from build123d import *

# Parameters (mm, degrees)
SKETCH_1_R          = 5.25
EXTRUDE_1_DEPTH     = 15
SKETCH_2_R          = 40
EXTRUDE_2_DEPTH     = 10
SKETCH_3_R          = 25
CUT_EXTRUDE_1_DEPTH = 113.805141727
FILLET_1_R          = 3


with BuildPart() as part:
    # 草图1 → 凸台-拉伸1 (new body)
    with BuildSketch(Plane.XY):
        with BuildLine():
            ThreePointArc((0, 77.781745931), (48.328171063, 48.328171063), (77.781745931, 0))
            ThreePointArc((77.781745931, 0), (48.328171063, -48.328171063), (0, -77.781745931))
            ThreePointArc((0, -77.781745931), (-48.328171063, -48.328171063), (-77.781745931, 0))
            ThreePointArc((-77.781745931, 0), (-48.328171063, 48.328171063), (0, 77.781745931))
        make_face()
        with Locations((0, 60)):
            Circle(SKETCH_1_R, mode=Mode.SUBTRACT)
        with Locations((60, 0)):
            Circle(SKETCH_1_R, mode=Mode.SUBTRACT)
        with Locations((0, -60)):
            Circle(SKETCH_1_R, mode=Mode.SUBTRACT)
        with Locations((-60, 0)):
            Circle(SKETCH_1_R, mode=Mode.SUBTRACT)
    extrude(amount=EXTRUDE_1_DEPTH)

    # 草图2 → 凸台-拉伸2 (add)
    with BuildSketch(Plane.XY.offset(15)):
        with Locations(Location((0, 0, 0), (0, 0, 180))):
            Circle(SKETCH_2_R)
    extrude(amount=EXTRUDE_2_DEPTH)

    # 草图3 → 切除-拉伸1 (cut, through all)
    with BuildSketch(Plane.XY.offset(25)):
        Circle(SKETCH_3_R)
    extrude(amount=-CUT_EXTRUDE_1_DEPTH, mode=Mode.SUBTRACT)

    # 圆角1
    fillet_1_edges = [part.edges().sort_by_distance(p)[0] for p in [
        (48.328171063, -48.328171063, 15),
        (48.328171063, 48.328171063, 15),
        (40, 0, 15),
        (40, 0, 25),
        (-48.328171063, 48.328171063, 15),
        (-48.328171063, -48.328171063, 15),
    ]]
    fillet(fillet_1_edges, radius=FILLET_1_R)


solid = part.part
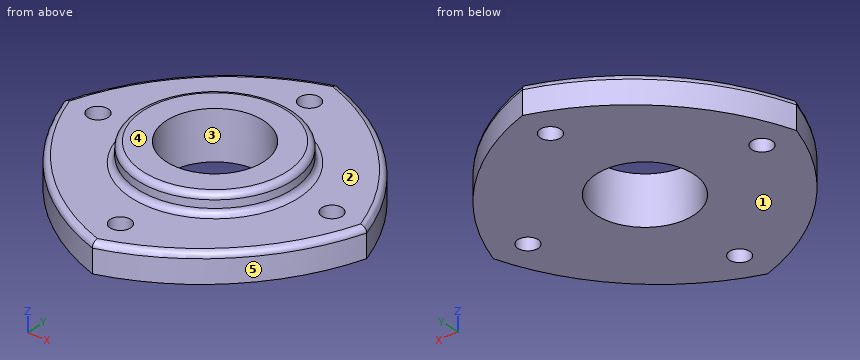
Input: part model. Units: mm. Frame: model coordinates. Face numbers are marked on the shaded views. A direction names the side the tool comes from. Round coordinates to 2 decimals unless told otherwise and drop trailing zeros. Order: outer loops, then holes, each group sorted by start corner. A loop starts at its lowest first (then second) coordinate and runs counter-clockwise, first axis right, second up. Notation, with made-up numbers: (57.5, 46) - (64.5, 46) arc R36 cw to (64.5, 85) - close; hole circle Ø2 at (-3.5, 22.5). An arc over 180 degrees is marked (long way). Answer as a JSON object with one key per item and string values. Group by question number.
(1) Reachability of the marked faces 1 and 2 from +Z, -Z, +X, -X, +Y, -Y: full face, straight path, thin tool, end or side. Return the list, or none.
(2) Draft query along X for the marked faces 3, 4 and 5. Return one class per face: released by +X, released by -X, zero draft, split by the parting line, or undercut.
(3) Material intervals for probe 1 along Y at (x, z) = (0, 10.25); probe 2 along Z at (x, y) = (-6, -66.5); probe 3 along X at (y, z) = (-22.5, 20.75), sorted ascending. Write a range as from..to.
(4) Pin query (flat end, axial travel): P1, Ø2, axis at x = -45, y = -15, coming from the -Z side; P2, Ø5, axis at y = -23.5, z = 18, coming from the -X side; P3, Ø2, axis at x = -4.5, z = 14, coming from the -Y side; P4, Ø12, axis at y = 41, z = 18.5, coming from the +X side. Return the tip coordinate at first contact, or that it passes through.
(5) Cut plane A-A (z = 7). Return loops of the section in (x, y).
Here are the results:
{
 "1": {"face 1": "-Z, +X, -X, +Y, -Y", "face 2": "+Z"},
 "2": {"face 3": "undercut", "face 4": "zero draft", "face 5": "released by +X"},
 "3": {"probe 1": "y = -77.78..-65.25, -54.75..-25, 25..54.75, 65.25..77.78", "probe 2": "z = 0..15", "probe 3": "x = -33.07..-10.9, 10.9..33.07"},
 "4": {"P1": "stops at z = 0", "P2": "stops at x = -34.35", "P3": "stops at y = -76.2", "P4": "stops at x = 57.34"},
 "5": {"outline": "(-77.78, 0) arc R120 ccw to (0, -77.78) arc R120 ccw to (77.78, 0) arc R120 ccw to (0, 77.78) arc R120 ccw to start; hole circle Ø10.5 at (-60, 0); hole circle Ø50 at (0, 0); hole circle Ø10.5 at (0, -60); hole circle Ø10.5 at (0, 60); hole circle Ø10.5 at (60, 0)"}
}
